Part model, mm, in its own coordinate system. A direction names the side the tool comes from. Round coordinates to 2 decimals unless told otherwise and drop trailing zeros. Write each loop counter-clockwise with the first axis right and the second up, starting at its lowest first coordinate (ties: lowest second). Pieces come first, ordered by that corner, then holes. Notation, with made-up numbers: M -26.5,-35.5 L -21.5,-35.5 A25 cw -21.5,-17.5 Z; hole C -24,5.5 d10. An arc over 180 degrees is marked long. Answer as a JSON object with one key per item and string values. Group by question number.
1. Band-saw the part on B-B, the plane x = 0. Write the cut outline in (y, z).
2. Band-saw the part on A-A, the plane z = 3.25. Write the cut outline in (x, y).
3. Which spindle directions (+Z, -Z, +X, -X, +Y, -Y) get a long thin tool onto all of the face, cutting with end or side? Do faces 4 (the face through (32, -18, 6)), 5 (the face through (23.846, 7.509, 3.944)). Say none if no direction does.
4. Drill centre lines: line 1 (Y direction, x = 0, z = 4.4); line 2 (X direction, y = 0.5, z = 6.75) (3 decimals); line 3 (X direction, y = 17.5, z = 3.25). Where is each one in solid material? Low to high. Write a range as from..to.
5. Two-plate mould, pull along Y, no slides. Class faces 1 (the face through (19, -19, 8)), 2 (the face through (20.765, -39.923, 3.944)), 3 (the face through (0, -37, 6)): +Y half, -Y half, draft (parallel to the pull), parting line (faces both ways), or undercut.
6. Band-saw the part on C-C, the plane y = -18.5. Write the cut outline in (x, z), plus the area to 3 significant figures.
7. Drop flat-ended pins along their axis: pin 1 (3 mm diameter, centred on y = -6, z = 2.5, fed in from +X); pin 2 (2.5 mm diameter, centred on x = -1, y = -36.5, fed in from -Z); pin 3 (1.5 mm diameter, centred on x = 5.5, z = 1, fed in from +Y). Give the stop position or say it passes through.
8. Band-saw the part on D-D, the plane y = -37. Write the cut outline in (x, z).
from build123d import *

# Parameters (mm, degrees)
SKETCH1_R           = 45
SKETCH1_R_2         = 25
BOSS_EXTRUDE1_DEPTH = 8
SKETCH2_R           = 42
SKETCH2_R_2         = 25
BOSS_EXTRUDE2_DEPTH = 3
SKETCH3_R           = 2.5
CUT_EXTRUDE1_DEPTH  = 6
CHAMFER1_SIZE       = 1
SKETCH4_R           = 42
SKETCH4_R_2         = 55
CUT_EXTRUDE2_DEPTH  = 3


with BuildPart() as part:
    # Sketch1 → Boss-Extrude1 (new body)
    with BuildSketch(Plane.XY):
        Circle(SKETCH1_R)
        Circle(SKETCH1_R_2, mode=Mode.SUBTRACT)
    extrude(amount=BOSS_EXTRUDE1_DEPTH)

    # Sketch2 → Boss-Extrude2 (add)
    with BuildSketch(Plane.XY.offset(8)):
        Circle(SKETCH2_R)
        Circle(SKETCH2_R_2, mode=Mode.SUBTRACT)
    extrude(amount=BOSS_EXTRUDE2_DEPTH)

    # Sketch3 → Cut-Extrude1 (cut)
    with BuildSketch(Plane(origin=(0, 0, 0), x_dir=(-1, 0, 0), z_dir=(0, 0, -1))):
        with Locations((0, 37)):
            Circle(SKETCH3_R)
        with Locations((32.04293994, 18.5)):
            Circle(SKETCH3_R)
        with Locations((32.04293994, -18.5)):
            Circle(SKETCH3_R)
        with Locations((0, -37)):
            Circle(SKETCH3_R)
        with Locations((-32.04293994, -18.5)):
            Circle(SKETCH3_R)
        with Locations((-32.04293994, 18.5)):
            Circle(SKETCH3_R)
    extrude(amount=-CUT_EXTRUDE1_DEPTH, mode=Mode.SUBTRACT)

    # Chamfer1
    chamfer1_edges = [part.edges().sort_by_distance(p)[0] for p in [
        (-42, 0, 11),
        (-25, 0, 11),
    ]]
    chamfer(chamfer1_edges, length=CHAMFER1_SIZE)

    # Sketch4 → Cut-Extrude2 (cut)
    with BuildSketch(Plane(origin=(248.99389391, -65.332745645, 8), x_dir=(0.8404902422792763, -0.5418266813597531, 0), z_dir=(0, 0, -1))):
        with Locations((-244.675962976, 80)):
            Circle(SKETCH4_R)
        with Locations((-244.675962976, -130)):
            Circle(SKETCH4_R_2)
    extrude(amount=-CUT_EXTRUDE2_DEPTH, mode=Mode.SUBTRACT)


solid = part.part
Worked answers:
{
 "1": {"outline": "M -45,0 L -39.5,0 L -39.5,6 L -34.5,6 L -34.5,0 L -25,0 L -25,8 L -45,8 Z; M 25,0 L 34.5,0 L 34.5,6 L 39.5,6 L 39.5,0 L 45,0 L 45,8 L 25,8 Z"},
 "2": {"outline": "C 0,0 d90; hole C -32.04,-18.5 d5; hole C -32.04,18.5 d5; hole C 0,0 d50; hole C 0,-37 d5; hole C 0,37 d5; hole C 32.04,-18.5 d5; hole C 32.04,18.5 d5"},
 "3": {"face 4": "-Z", "face 5": "+Z, -Z"},
 "4": {"line 1": "y = -45..-39.5, -34.5..-25, 25..34.5, 39.5..45", "line 2": "x = -44.997..-24.995, 24.995..44.997", "line 3": "x = -41.46..-34.33, -29.75..-17.85, 17.85..29.75, 34.33..41.46"},
 "5": {"face 1": "draft", "face 2": "parting line", "face 3": "undercut"},
 "6": {"outline": "M -41.02,0 L -34.54,0 L -34.54,6 L -29.54,6 L -29.54,0 L -16.82,0 L -16.82,8 L -41.02,8 Z; M 16.82,0 L 29.54,0 L 29.54,6 L 34.54,6 L 34.54,0 L 41.02,0 L 41.02,8 L 16.82,8 Z", "area": "327 mm^2"},
 "7": {"pin 1": "stops at x = 44.77", "pin 2": "stops at z = 6", "pin 3": "stops at y = 44.75"},
 "8": {"outline": "M -25.61,0 L -2.5,0 L -2.5,6 L 2.5,6 L 2.5,0 L 25.61,0 L 25.61,8 L -25.61,8 Z"}
}
